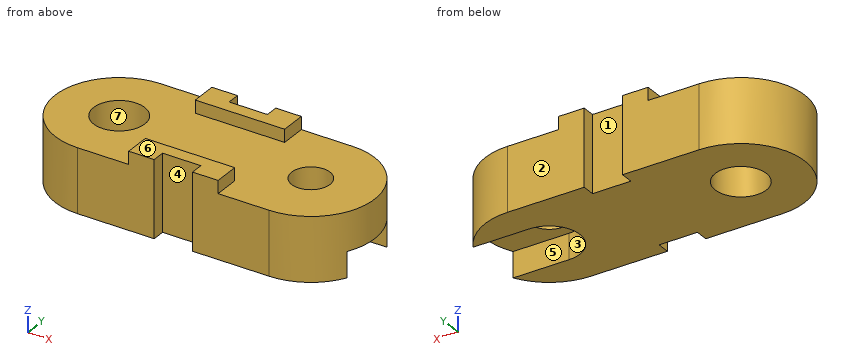
```python
from build123d import *

# Parameters (mm, degrees)
LINK_BODY_DEPTH       = 25
SIDE_PADS_35X10_DEPTH = 5
T_SLOTS_DEPTH         = 35
CROSS_SLOT_12MM_DEPTH = 10
EYE_BORE_20_SKETCH_R  = 10
EYE_BORE_20_DEPTH     = 32
EYE_BORE_15_SKETCH_R  = 7.5
EYE_BORE_15_DEPTH     = 32


with BuildPart() as part:
    # Link Profile Sketch → Link Body (new body)
    with BuildSketch(Plane.XY):
        with BuildLine():
            Line((-37.5, 25), (37.5, 25))
            ThreePointArc((37.5, 25), (62.5, 0), (37.5, -25))
            Line((37.5, -25), (-37.5, -25))
            ThreePointArc((-37.5, -25), (-62.5, 0), (-37.5, 25))
        make_face()
    extrude(amount=LINK_BODY_DEPTH)

    # Side Pads Sketch → Side Pads 35x10 (add)
    with BuildSketch(Plane.XY.offset(25)):
        Polygon((0, -15), (17.5, -15), (17.5, -25), (-17.5, -25), (-17.5, -15), align=None)
        Polygon((-17.5, 15), (0, 15), (17.5, 15), (17.5, 25), (-17.5, 25), align=None)
    extrude(amount=SIDE_PADS_35X10_DEPTH)

    # T-Slots Sketch → T-Slots (cut)
    with BuildSketch(Plane.XY.offset(30)):
        Polygon((0, -20), (7.5, -20), (7.5, -26.538654193), (-7.5, -26.538654193), (-7.5, -20), align=None)
        Polygon((-7.5, 20), (0, 20), (7.5, 20), (7.5, 26.538654193), (-7.5, 26.538654193), align=None)
    extrude(amount=-T_SLOTS_DEPTH, mode=Mode.SUBTRACT)

    # Cross Slot Sketch → Cross Slot 12mm (cut)
    with BuildSketch(Plane(origin=(0, 0, 0), x_dir=(-1, 0, 0), z_dir=(0, 0, -1))):
        with BuildLine():
            Line((-37.5, 12), (-67.446025863, 12))
            Line((-67.446025863, 12), (-67.446025863, -12))
            Line((-67.446025863, -12), (-37.5, -12))
            ThreePointArc((-37.5, -12), (-25.5, 0), (-37.5, 12))
        make_face()
    extrude(amount=-CROSS_SLOT_12MM_DEPTH, mode=Mode.SUBTRACT)

    # Eye Bore Ø20 Sketch → Eye Bore Ø20 (cut)
    with BuildSketch(Plane.XY.offset(25)):
        with Locations((-37.5, 0)):
            Circle(EYE_BORE_20_SKETCH_R)
    extrude(amount=-EYE_BORE_20_DEPTH, mode=Mode.SUBTRACT)

    # Eye Bore Ø15 Sketch → Eye Bore Ø15 (cut)
    with BuildSketch(Plane.XY.offset(25)):
        with Locations((37.5, 0)):
            Circle(EYE_BORE_15_SKETCH_R)
    extrude(amount=-EYE_BORE_15_DEPTH, mode=Mode.SUBTRACT)


solid = part.part
```
Geometry check sheet. Reference: the model listing, model coordinates, mm. Face numbers are marked on the shaded views. A direction names the side the tool comes from. Coordinates: 2 decimals unless noted, no trailing zeros. Order: outer loops, then holes, each group sorted by start corner. A loop starts at its lowest first (then second) coordinate and runs counter-clockwise, first axis right, second up.
Q1. Depth check by flat-ended pin: pin 1 Ø7.5 at (x, z) = (-3.5, 14) entering from +Y; pin 2 Ø4 at (y, z) = (-22.5, 18.5) entering from -X; pin 3 Ø1.5 at (y, z) = (-20.5, 27) entering from +X; pin 4 Ø12 at (x, y) = (37.5, 0) entering from -Z. Enter the tip coordinate at first touch or a pass-through.
Reply:
pin 1: stops at y = 20
pin 2: stops at x = -51.81
pin 3: stops at x = 17.5
pin 4: passes through
Q2. Sectioned sample at D-D on x = 12.5. Record the cut outline in (y, z).
Reply:
outline: (-25, 0) - (25, 0) - (25, 30) - (15, 30) - (15, 25) - (-15, 25) - (-15, 30) - (-25, 30) - close
Q3. Sectioned sample at C-C on z = 26.75. Record the cut outline in (x, y), and give its area (3 significant figures).
Reply:
outline: (-17.5, -25) - (-7.5, -25) - (-7.5, -20) - (7.5, -20) - (7.5, -25) - (17.5, -25) - (17.5, -15) - (-17.5, -15) - close; (-17.5, 15) - (17.5, 15) - (17.5, 25) - (7.5, 25) - (7.5, 20) - (-7.5, 20) - (-7.5, 25) - (-17.5, 25) - close
area: 550 mm2
Q4. Tool access check on the marked faces 1, 2 and 3. Record the directions out of +Z, -Z, +X, -X, +Y, -Y that give a thin tool (end or side, any length) a straight path to the whole face; none if there is none.
Reply:
face 1: +Z, -Z, +Y
face 2: +Z, -Z, +X, -X, +Y
face 3: -Z, +X
Q5. Thickness scan on probe 1 along X at (y, z) = (-0.5, 20) (1 decimal); probe 2 along Y at (x, z) = (37.5, 15); probe 3 along Z at (x, y) = (44, -10). Record the ranges inside material, lowest first.
Reply:
probe 1: x = -62.5 to -47.5, -27.5 to 30, 45 to 62.5
probe 2: y = -25 to -7.5, 7.5 to 25
probe 3: z = 10 to 25
Q6. Sectioned sample at B-B on y = 0. Record the cut outline in (x, z).
Reply:
outline: (-62.5, 0) - (-47.5, 0) - (-47.5, 25) - (-62.5, 25) - close; (-27.5, 0) - (25.5, 0) - (25.5, 10) - (30, 10) - (30, 25) - (-27.5, 25) - close; (45, 10) - (62.5, 10) - (62.5, 25) - (45, 25) - close
Q7. Sectioned sample at A-A on z = 11.5. Record the cut outline in (x, y).
Reply:
outline: (-37.5, -25) - (-7.5, -25) - (-7.5, -20) - (7.5, -20) - (7.5, -25) - (37.5, -25) arc R25 ccw to (37.5, 25) - (7.5, 25) - (7.5, 20) - (-7.5, 20) - (-7.5, 25) - (-37.5, 25) arc R25 ccw to start; hole circle Ø20 at (-37.5, 0); hole circle Ø15 at (37.5, 0)
Q8. Draft check along Y on the marked faces 4, 5, 6 and 7. Enter one of: released by +Y, released by -Y, zero draft, split by the parting line, or undercut.
Reply:
face 4: released by -Y
face 5: undercut
face 6: zero draft
face 7: undercut
